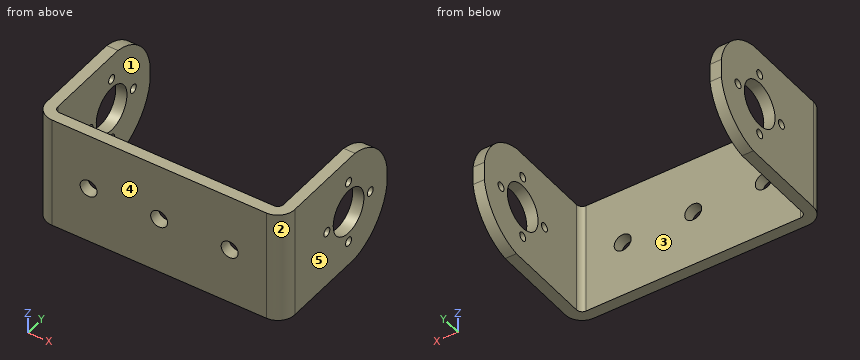
from build123d import *

# Parameters (mm, degrees)
BOSS_EXTRUDE1_DEPTH = 20
SKETCH2_R           = 4
SKETCH2_R_2         = 0.771303816
CUT_EXTRUDE1_DEPTH  = 55.415071442
SKETCH3_R           = 1.5
CUT_EXTRUDE2_DEPTH  = 53.810983706


with BuildPart() as part:
    # Sketch1 → Boss-Extrude1 (new body)
    with BuildSketch(Plane.XY):
        with BuildLine():
            Line((0, 25), (0, 1))
            ThreePointArc((0, 1), (0.292893219, 0.292893219), (1, 0))
            Line((1, 0), (39, 0))
            ThreePointArc((39, 0), (39.707106781, 0.292893219), (40, 1))
            Line((40, 1), (40, 25))
            Line((40, 25), (42, 25))
            Line((42, 25), (42, 1))
            ThreePointArc((42, 1), (41.121320344, -1.121320344), (39, -2))
            Line((39, -2), (1, -2))
            ThreePointArc((1, -2), (-1.121320344, -1.121320344), (-2, 1))
            Line((-2, 1), (-2, 25))
            Line((-2, 25), (0, 25))
        make_face()
    extrude(amount=BOSS_EXTRUDE1_DEPTH)

    # Sketch2 → Cut-Extrude1 (cut, through all)
    with BuildSketch(Plane.ZY.offset(2)):
        with Locations((10, 15)):
            Circle(SKETCH2_R)
        with Locations((10, 20.651236345)):
            Circle(SKETCH2_R_2)
        with Locations((15.651236345, 15)):
            Circle(SKETCH2_R_2)
        with Locations((10, 9.348763655)):
            Circle(SKETCH2_R_2)
        with Locations((4.348763655, 15)):
            Circle(SKETCH2_R_2)
        with BuildLine():
            Line((-0.134788382, 15), (-9.479992385, 25.134788382))
            Line((-9.479992385, 25.134788382), (9.199881334, 33.71105644))
            Line((9.199881334, 33.71105644), (31.219173818, 26.927862072))
            Line((31.219173818, 26.927862072), (20.134788382, 15))
            ThreePointArc((20.134788382, 15), (10, 25.134788382), (-0.134788382, 15))
        make_face()
    extrude(amount=-CUT_EXTRUDE1_DEPTH, mode=Mode.SUBTRACT)

    # Sketch3 → Cut-Extrude2 (cut, through all)
    with BuildSketch(Plane(origin=(0, 0, 0), x_dir=(1, 0, 0), z_dir=(0, 1, 0))):
        with Locations(Location((7.5, -10, 0), (0, 0, 270))):
            Circle(SKETCH3_R)
        with Locations(Location((20, -10, 0), (0, 0, 270))):
            Circle(SKETCH3_R)
        with Locations(Location((32.5, -10, 0), (0, 0, 270))):
            Circle(SKETCH3_R)
    extrude(amount=-CUT_EXTRUDE2_DEPTH, mode=Mode.SUBTRACT)


solid = part.part
The model under review builds one solid part; all positions refer to its coordinate system, in mm. Face numbers are marked on the shaded views. A direction names the side the tool comes from. Round coordinates to 2 decimals unless told otherwise and drop trailing zeros. Order: outer loops, then holes, each group sorted by start corner. A loop starts at its lowest first (then second) coordinate and runs counter-clockwise, first axis right, second up. Notation, with made-up numbers: (8.25, -3.5) -> (25.25, -3.5) arc R17 ccw to (25.25, 14.5) -> close; hole circle Ø2 at (42.5, 64). An arc over 180 degrees is marked (long way). Write item = value, one per line. Start each with the question number.
Item 1: Mouldability with a two-part tool opening along X and no side actions: class the marked faces 3, 4 and 5 as released by +X, released by -X, zero draft, split by the parting line, or undercut.
Item 2: For line 1 along X through (y, z) = (22, 15); line 2 along X through (y, z) = (-1, 10); line 3 along Y through (x, z) = (41.5, 10), list the stretches that pass through material, from the lowest coordinate up.
Item 3: Consider section A-A on x = 32.5. Write out the cut boundary in (y, z).
Item 4: For the marked faces 1 and 2, list the 3-axis set-ups (+Z, -Z, +X, -X, +Y, -Y) from which the entire face can be reached by the end or side of a thin tool; tool diameter is ignored.
Item 5: Clearance check with a flat-ended pin moving along its axis: pin 1 Ø10 at (x, z) = (28, 14.5) entering from +Y. State where the tip first meets the part, or that it passes through.
Item 6: Consider section D-D on x = 24.5. Write out the cut boundary in (y, z), plus the area to 3 significant figures.
Item 7: Consider section C-C on z = 17.5. Write out the cut boundary in (x, y).
Item 8: Consider section B-B on z = 10. Count the separate pieces of the cut face and the enclosed holes in it, plus the area to 3 significant figures.
Conclusion:
q1.face_3 = undercut
q1.face_4 = zero draft
q1.face_5 = released by +X
q2.line_1 = -2 to 0, 40 to 42
q2.line_2 = -1.24 to 6, 9 to 18.5, 21.5 to 31, 34 to 41.24
q2.line_3 = -0.66 to 8.58, 10.12 to 11, 19 to 19.88, 21.42 to 25
q3.outline = (-2, 0) -> (0, 0) -> (0, 8.5) -> (-2, 8.5) -> close; (-2, 11.5) -> (0, 11.5) -> (0, 20) -> (-2, 20) -> close
q4.face_1 = +Z, -Z, +Y
q4.face_2 = +Z, -Z, +X, -Y
q5.pin_1 = 0
q6.outline = (-2, 0) -> (0, 0) -> (0, 20) -> (-2, 20) -> close
q6.area = 40.0 mm2
q7.outline = (-2, 1) arc R3 ccw to (1, -2) -> (39, -2) arc R3 ccw to (42, 1) -> (42, 21.82) -> (40, 21.82) -> (40, 1) arc R1 cw to (39, 0) -> (1, 0) arc R1 cw to (0, 1) -> (0, 21.82) -> (-2, 21.82) -> close
q8.separate_pieces = 10
q8.enclosed_holes = 0
q8.area = 122 mm2
